Design review of the part built by this model. Coordinates are the model's own, in mm. A direction names the side the tool comes from. Give positions to 0.01 mm unless a question says otherwise; leave off trailing zeros. Loops run counter-clockwise (first coordinate to the right, second up) from the corner with the lowest first, then second, coordinate; pieces in that order, holes last. Notation, with made-up numbers: M -9.75,-17.5 L 24.25,-17.5 A18 ccw 24.25,10.5 Z; hole C -2,60.25 d11. An arc over 180 degrees is marked long. Use one line per item in the form item = value. Start each with the question number.
from build123d import *

# Parameters (mm, degrees)
EXTRUDE_1_DEPTH         = 1150
HOLE_WIZARD_12_0_12_1_D = 12
SKETCH_4_W              = 30
SKETCH_4_H              = 50.480703337
CUT_EXTRUDE_1_DEPTH     = 10


with BuildPart() as part:
    # 草图1 → 拉伸1 (new body)
    with BuildSketch(Plane.XY):
        with BuildLine():
            Line((0, 0), (0, 40))
            Line((0, 40), (3.99, 40))
            ThreePointArc((3.99, 40), (3.997071068, 39.997071068), (4, 39.99))
            Line((4, 39.99), (4, 9))
            ThreePointArc((4, 9), (5.464466094, 5.464466094), (9, 4))
            Line((9, 4), (39.99, 4))
            ThreePointArc((39.99, 4), (39.997071068, 3.997071068), (40, 3.99))
            Line((40, 3.99), (40, 0))
            Line((40, 0), (0, 0))
        make_face()
    extrude(amount=EXTRUDE_1_DEPTH)

    # Ø12.0 (12) 直径孔1 (through all)
    with Locations(Plane(origin=(0, 4, 0), x_dir=(1, 0, 0), z_dir=(0, 1, 0))):
        with Locations((24.99, -1132), (24.99, -614), (24.99, -536), (24.99, -18)):
            Hole(HOLE_WIZARD_12_0_12_1_D / 2)

    # 草图4 → 切除-拉伸1 (cut)
    with BuildSketch(Plane(origin=(4, 0, 0), x_dir=(0, 0, -1), z_dir=(1, 0, 0))):
        with Locations((-575, 35.240351668)):
            Rectangle(SKETCH_4_W, SKETCH_4_H)
    extrude(amount=-CUT_EXTRUDE_1_DEPTH, mode=Mode.SUBTRACT)


solid = part.part
Q1. Wall thickness on probe 1 along Z at (x, y) = (24, 1); probe 2 along Z at (x, y) = (24.99, 1); probe 3 along X at (y, z) = (2.35, 614): over which ranges is each line inside the solid? List them lowest first.
Q2. Take a section at B-B on y = 32.5. Give the boundary of the cut face in (x, z), plus the area to 3 significant figures.
Q3. For faces 1 (the flat face through (24, 4, 567)), 2 (the flat face through (20, 0, 567)), list the 3-axis set-ups (+Z, -Z, +X, -X, +Y, -Y) from which the entire face can be reached by the end or side of a thin tool; tool diameter is ignored.
Q4. Clearance check with flat-ended pins moving along their axes: pin 1 Ø1.2 at (x, z) = (2.5, 579.5) entering from +Y; pin 2 Ø9.5 at (x, z) = (32, 481.5) entering from +Y; pin 3 Ø8 at (y, z) = (29.5, 781.5) entering from +X. State where each tip first meets the part, or that it passes through.
Q5. Take a section at A-A on x = 24.99. Give the boundary of the cut face in (y, z).
Response values:
q1.probe_1 = 0 to 12.08, 23.92 to 530.08, 541.92 to 608.08, 619.92 to 1126.08, 1137.92 to 1150
q1.probe_2 = 0 to 12, 24 to 530, 542 to 608, 620 to 1126, 1138 to 1150
q1.probe_3 = 0 to 18.99, 30.99 to 40
q2.outline = M 0,0 L 4,0 L 4,560 L 0,560 Z; M 0,590 L 4,590 L 4,1150 L 0,1150 Z
q2.area = 4,480 mm^2
q3.face_1 = +Z, -Z, +X, +Y
q3.face_2 = +Z, -Z, +X, -X, -Y
q4.pin_1 = 10
q4.pin_2 = 4
q4.pin_3 = 4
q5.outline = M 0,0 L 4,0 L 4,12 L 0,12 Z; M 0,24 L 4,24 L 4,530 L 0,530 Z; M 0,542 L 4,542 L 4,608 L 0,608 Z; M 0,620 L 4,620 L 4,1126 L 0,1126 Z; M 0,1138 L 4,1138 L 4,1150 L 0,1150 Z
